Here's the drawing with two shaded views (mm, measured from the low corner). I have some questions. A direction names the side the tool comes from. Round coordinates to 2 decimals unless told otherwise and drop trailing zeros. Write each loop counter-clockwise with the first axis right and the second up, starting at its lowest first coordinate (ties: lowest second). Pieces come first, ordered by that corner, then holes. Notation, with made-up numbers: (1.5, 64) -> (36.5, 64) arc R3 cw to (36.5, 68) -> close; hole circle Ø3 at (78.5, -23.5). An arc over 180 degrees is marked (long way). Use CSV: the item, a comma, the result in double quotes.
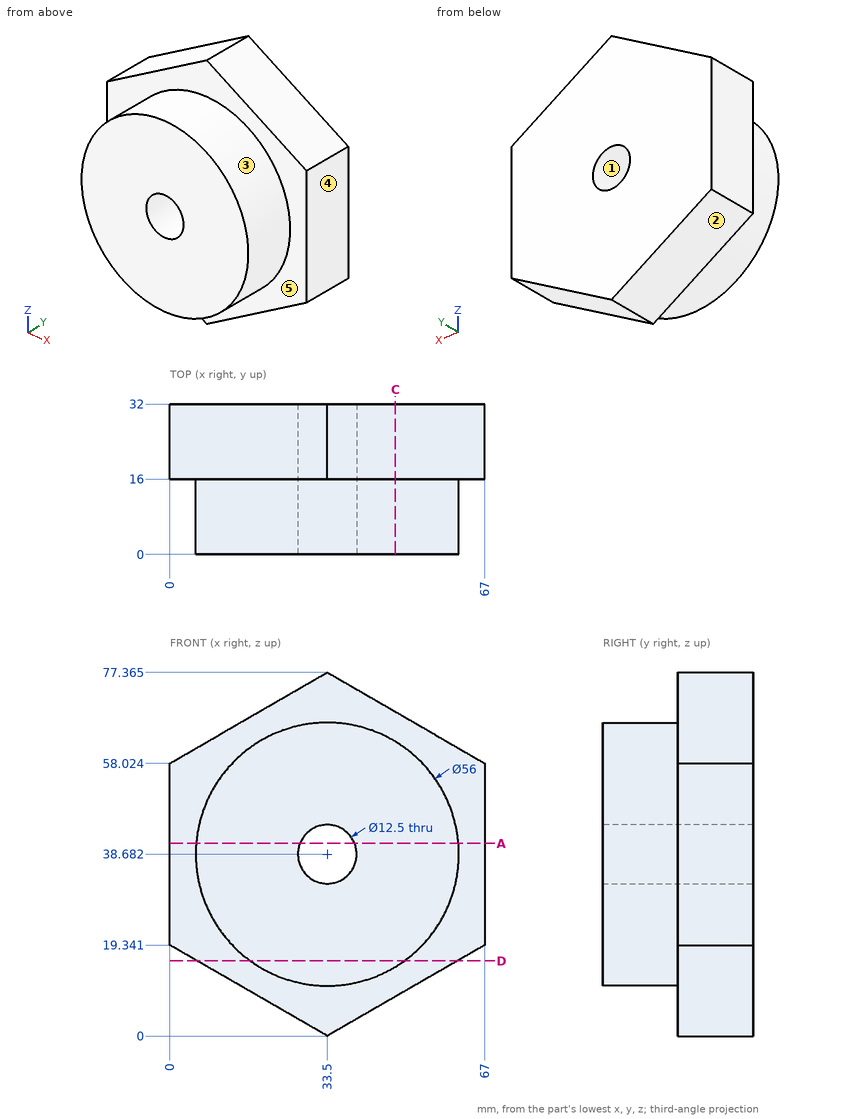
Q1. Suppose I cut it at D-D (z = 16). Write out the boundary of the cut face in (x, y), and give its area (3 significant figures).
Resolved:
outline,"(5.79, 16) -> (17.08, 16) -> (17.08, 0) -> (49.92, 0) -> (49.92, 16) -> (61.21, 16) -> (61.21, 32) -> (5.79, 32) -> close"
area,"1,410 mm^2"
Q2. Will these pins go through, and if not, where does the flat tip stop? P1, Ø5, axis at y = 4, z = 41, coming from the +X side; P2, Ø5, axis at x = 9, y = 23, coming from the -Z side.
Resolved:
P1,"stops at x = 61.5"
P2,"stops at z = 12.7"
Q3. Suppose I cut it at C-C (x = 48). Write out the boundary of the cut face in (y, z) (1 decimal).
Resolved:
outline,"(0, 14.7) -> (16, 14.7) -> (16, 8.4) -> (32, 8.4) -> (32, 69) -> (16, 69) -> (16, 62.6) -> (0, 62.6) -> close"
Q4. On a 3-axis mill with a long thin cutter (end or side, diameter ignored), from which of +Z, -Z, +X, -X, +Y, -Y can I reach the whole of each face in a straight line? I mean the marked faces 4 and 5. Say none if no direction works.
Resolved:
face 4,"+Z, -Z, +X, +Y, -Y"
face 5,"-Y"
Q5. Suppose I cut it at A-A (z = 41). Write out the boundary of the cut face in (x, y) (1 decimal), and give its area (3 significant figures).
Resolved:
outline,"(0, 16) -> (5.6, 16) -> (5.6, 0) -> (27.7, 0) -> (27.7, 32) -> (0, 32) -> close; (39.3, 0) -> (61.4, 0) -> (61.4, 16) -> (67, 16) -> (67, 32) -> (39.3, 32) -> close"
area,"1,590 mm^2"
Q6. If we mould it in two halves opening along Z, with no side actions, what happens to the marked faces 1, 2 and 3? For each: released by +Z, released by -Z, zero draft, split by the parting line, or undercut.
Resolved:
face 1,"undercut"
face 2,"released by -Z"
face 3,"split by the parting line"
Q7. Please list where these lines run through material, in increasing order: probe 1 along Z at (x, y) = (33, 12); probe 2 along Y at (x, z) = (43, 70.5); probe 3 along X at (y, z) = (26, 39.5).
Resolved:
probe 1,"z = 10.69 to 32.45, 44.91 to 66.68"
probe 2,"y = 16 to 32"
probe 3,"x = 0 to 27.3, 39.7 to 67"
